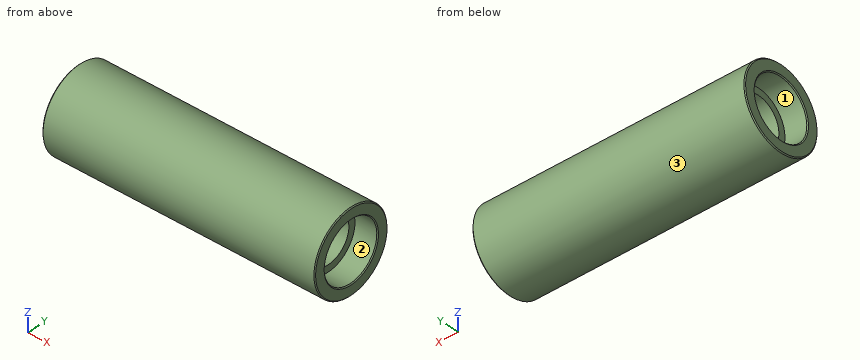
from build123d import *

# Parameters (mm, degrees)
CHAMFER1_SIZE = 0.2


with BuildPart() as part:
    # Sketch1 → Revolve1 (revolve)
    with BuildSketch(Plane.XY, mode=Mode.PRIVATE) as revolve1_sk:
        Polygon((0, 9), (60, 9), (60, 6.5), (55, 6.5), (55, 5), (5, 5), (5, 6.5), (0, 6.5), align=None)
    revolve(revolve1_sk.sketch.rotate(Axis((0, 0, 0), (1, 0, 0)), 90), axis=Axis((0, 0, 0), (1, 0, 0)))

    # Chamfer1
    chamfer1_edges = [part.edges().sort_by_distance(p)[0] for p in [
        (0, 0, -6.5),
        (60, 0, -6.5),
        (60, 0, -9),
        (0, 0, -9),
    ]]
    chamfer(chamfer1_edges, length=CHAMFER1_SIZE)


solid = part.part
Could you check a few things on this model? Use its own coordinates, in mm. Face numbers are marked on the shaded views. A direction names the side the tool comes from. Round coordinates to 2 decimals unless told otherwise and drop trailing zeros. Write each loop counter-clockwise with the first axis right and the second up, starting at its lowest first coordinate (ties: lowest second). Pieces come first, ordered by that corner, then holes. Notation, with made-up numbers: (14.25, 83) - (47.25, 83) arc R13 ccw to (47.25, 90) - close; hole circle Ø4 at (71.25, -20). An arc over 180 degrees is marked (long way). Put each result on its own line as item: value. Start each with the question number.
(1) I want a section at A-A, the plane y = 0. Please give me the cut outline in (x, z), plus the area to 3 significant figures.
(2) For the marked faces 1, 2 and 3, which set-ups out of +Z, -Z, +X, -X, +Y, -Y let a thin tool reach every point of the face, with its end or its side?
(3) Will these pins go through, and if not, where does the flat tip stop? pin 1 (8 mm diameter, centred on y = 0, z = 0, fed in from -X); pin 2 (6.5 mm diameter, centred on y = 0.5, z = 3, fed in from +X); pin 3 (1.5 mm diameter, centred on x = 46.5, y = -1, fed in from -Z); pin 4 (1.5 mm diameter, centred on x = 13.5, z = -5.5, fed in from -Y).
(4) I need wall thicknesses on probe 1 along Y at (x, z) = (42, 0); probe 2 along Y at (x, z) = (1.4, 0); probe 3 along Z at (x, y) = (3, 3.5). Which ranges of each line are inside material? Lowest first, please.
(5) I want a section at C-C, the plane x = 39. Please give me the cut outline in (y, z), plus the area to 3 significant figures.
Here are the results:
1. outline: (0, -8.8) - (0.2, -9) - (59.8, -9) - (60, -8.8) - (60, -6.7) - (59.8, -6.5) - (55, -6.5) - (55, -5) - (5, -5) - (5, -6.5) - (0.2, -6.5) - (0, -6.7) - close; (0, 6.7) - (0.2, 6.5) - (5, 6.5) - (5, 5) - (55, 5) - (55, 6.5) - (59.8, 6.5) - (60, 6.7) - (60, 8.8) - (59.8, 9) - (0.2, 9) - (0, 8.8) - close
1. area: 450 mm^2
2. face 1: -X
2. face 2: +X
2. face 3: +X, -X
3. pin 1: passes through
3. pin 2: stops at x = 55
3. pin 3: stops at z = -9
3. pin 4: stops at y = -7.64
4. probe 1: y = -9 to -5, 5 to 9
4. probe 2: y = -9 to -6.5, 6.5 to 9
4. probe 3: z = -8.29 to -5.48, 5.48 to 8.29
5. outline: circle Ø18 at (0, 0); hole circle Ø10 at (0, 0)
5. area: 176 mm^2
